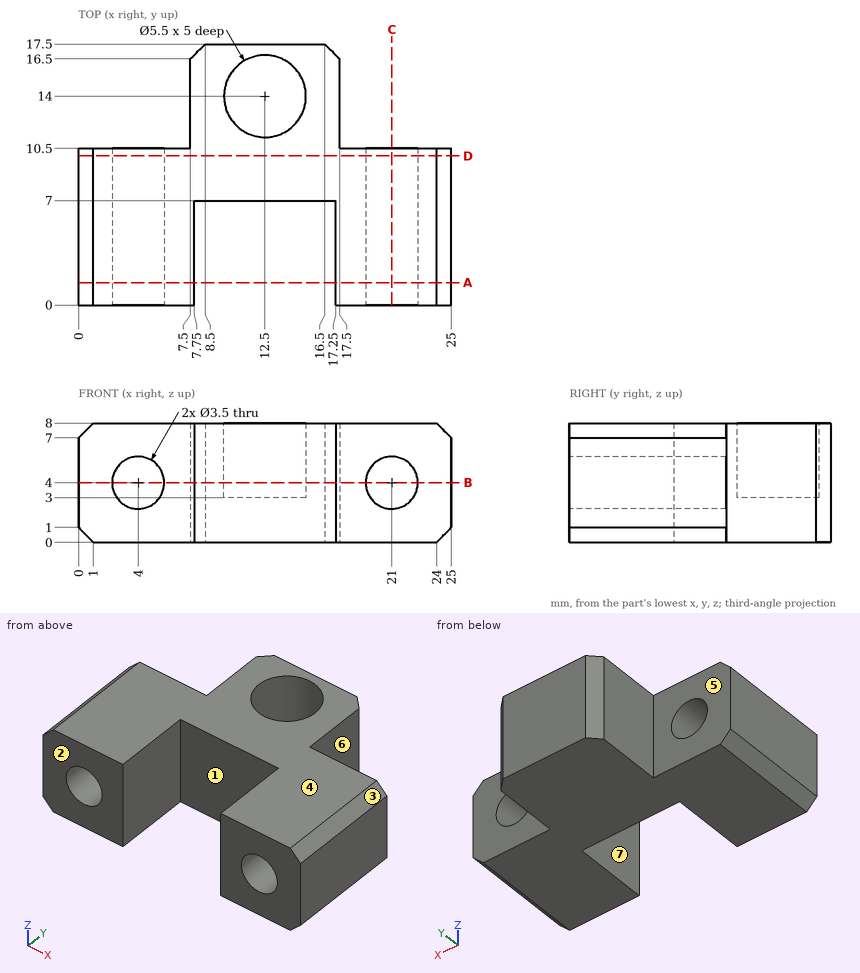
Job drawing, mm, ordinate dimensions from the low corner. One solid piece. A direction names the side the tool comes from. Round coordinates to 2 decimals unless told otherwise and drop trailing zeros. Loops run counter-clockwise (first coordinate to the right, second up) from the corner with the lowest first, then second, coordinate; pieces in that order, holes last.
(1) Wall check: line 1 along X through (y, z) = (4.75, 4); line 2 along X through (y, z) = (5.5, 1.75); line 3 along Z through (x, y) = (21, 7.75). Give the ranges that are in metal, low to high.
(2) Cut at A-A (y = 1.5). Give the cut face in (x, z).
(3) Which spindle directions (+Z, -Z, +X, -X, +Y, -Y) get a long thin tool onto all of the face, cutting with end or side? Do the marked faces 4, 5, 6 and 7. Say none if no direction does.
(4) Two-plate mould, pull along X, no slides. Class the marked faces 1, 2 and 3: +X half, -X half, draft (parallel to the pull), parting line (faces both ways), or undercut.
(5) Cut at D-D (y = 10). Give the cut face in (x, z).
(6) Cut at B-B (z = 4). Give the cut face in (x, y).
(7) Cut at C-C (x = 21). Give the cut face in (y, z).
(8) Drop flat-ended pins along their axis: pin 1 (6 mm diameter, centred on x = 11.5, y = 13, fed in from +Z); pin 2 (2 mm diameter, centred on x = 23, z = 2, fed in from +Y); pin 3 (3 mm diameter, centred on x = 21, z = 4, fed in from +Y); pin 4 (4 mm diameter, centred on x = 14.5, z = 5.5, fed in from -Y). Give the stop position or say it passes through.
Findings below:
1. line 1: x = 0 to 2.25, 5.75 to 7.75, 17.25 to 19.25, 22.75 to 25
1. line 2: x = 0 to 7.75, 17.25 to 25
1. line 3: z = 0 to 2.25, 5.75 to 8
2. outline: (0, 1) - (1, 0) - (7.75, 0) - (7.75, 8) - (1, 8) - (0, 7) - close; (17.25, 0) - (24, 0) - (25, 1) - (25, 7) - (24, 8) - (17.25, 8) - close; hole circle Ø3.5 at (4, 4); hole circle Ø3.5 at (21, 4)
3. face 4: +Z, +X, -X, +Y, -Y
3. face 5: +Z, -Z, -X, +Y
3. face 6: +Z, -Z, +X, +Y
3. face 7: +Z, -Z, -Y
4. face 1: undercut
4. face 2: draft
4. face 3: +X half
5. outline: (0, 1) - (1, 0) - (24, 0) - (25, 1) - (25, 7) - (24, 8) - (1, 8) - (0, 7) - close; hole circle Ø3.5 at (4, 4); hole circle Ø3.5 at (21, 4)
6. outline: (0, 0) - (2.25, 0) - (2.25, 10.5) - (0, 10.5) - close; (5.75, 0) - (7.75, 0) - (7.75, 7) - (17.25, 7) - (17.25, 0) - (19.25, 0) - (19.25, 10.5) - (17.5, 10.5) - (17.5, 16.5) - (16.5, 17.5) - (8.5, 17.5) - (7.5, 16.5) - (7.5, 10.5) - (5.75, 10.5) - close; (22.75, 0) - (25, 0) - (25, 10.5) - (22.75, 10.5) - close; hole circle Ø5.5 at (12.5, 14)
7. outline: (0, 0) - (10.5, 0) - (10.5, 2.25) - (0, 2.25) - close; (0, 5.75) - (10.5, 5.75) - (10.5, 8) - (0, 8) - close
8. pin 1: stops at z = 8
8. pin 2: stops at y = 10.5
8. pin 3: passes through
8. pin 4: stops at y = 7
